Check sheet for the modelled part. Datum: model origin and axes. Units: mm. Give positions to 0.01 mm unless a question says otherwise; leave off trailing zeros. Loops run counter-clockwise (first coordinate to the right, second up) from the corner with the lowest first, then second, coordinate; pieces in that order, holes last. Notation, with made-up numbers: (-10, 45.25) -> (48, 45.25) arc R30 ccw to (48, 78.25) -> close; hole circle Ø8 at (69, 12). An arc over 180 degrees is marked (long way). Answer as CSV lines item,"result". Start each with the question number.
(1) Gauge pin test, flat ends, axial feed: pin 1 Ø1.5 at (y, z) = (214, 5) entering from -X; pin 2 Ø2 at (x, z) = (170, 4) entering from +Y; pin 3 Ø2 at (y, z) = (125.5, 5.5) entering from +X. Record the tip position at first contact, or that the pin passes through.
(2) Material ranges on line 1 (X direction, y = 262, z = 6); line 2 (Y direction, x = 0, z = 3); line 3 (Y direction, x = 20.5, z = 4.5), recorded low to high. Write a range as from..to.
(3) Section check B-B on x = 67. Enter the section's corners in (y, z).
(4) Release check for a two-part mould opening along Y. For faces 1 (the face through (7.917, 143.864, 4.93)), 2 (the face through (193.65, 258.174, 4.93)), 3 (the face through (44, 152, 5)), 4 (the face through (200.4, 252.26, 4.93)) record: pulls with the +Y half, pulls with the -Y half, needs draft (parallel to the pull), parting line crosses it, or undercut.
(5) Section check C-C on y = 219. Enter the section's corners in (x, z), plus the area to 3 significant figures.
(6) Section check A-A on z = 6.25. State how many separate pieces and enclosed holes the cut face has, plus the area to 3 significant figures.
from build123d import *

# Parameters (mm, degrees)
SKETCH_1_R      = 3
SKETCH_1_R_2    = 16
SKETCH_1_R_3    = 3.91899873
SKETCH_1_R_4    = 2
EXTRUDE_1_DEPTH = 10


with BuildPart() as part:
    # 草图1 → 凸台-拉伸1 (new body)
    with BuildSketch(Plane.XY):
        with BuildLine():
            Line((-14, 128), (-6, 0))
            ThreePointArc((-6, 0), (0, -6), (6, 0))
            add(Edge.make_bspline(
                [(6, 0), (1.588652615, 45.680929706), (5.604102499, 79.643200211), (28.004797731, 112.13093391)],
                knots=[0, 0, 0, 0, 0.788155359, 0.788155359, 0.788155359, 0.788155359], degree=3))
            ThreePointArc((28.004797731, 112.13093391), (50.113637924, 128.900750568), (77, 135.767416406))
            ThreePointArc((77, 135.767416406), (157.787149523, 170.485384951), (196.379869136, 249.494896157))
            ThreePointArc((196.379869136, 249.494896157), (200.439238403, 252.311917913), (202, 257))
            Line((202, 257), (202, 262))
            ThreePointArc((202, 262), (194.5, 269.5), (187, 262))
            ThreePointArc((187, 262), (154.781745931, 184.218254069), (77, 152))
            Line((77, 152), (10, 152))
            ThreePointArc((10, 152), (-6.970562748, 144.970562748), (-14, 128))
        make_face()
        Circle(SKETCH_1_R, mode=Mode.SUBTRACT)
        with Locations((10, 128)):
            Circle(SKETCH_1_R_2, mode=Mode.SUBTRACT)
        with Locations((194.5, 262)):
            Circle(SKETCH_1_R_3, mode=Mode.SUBTRACT)
        with Locations((0, 12.5)):
            Circle(SKETCH_1_R_4, mode=Mode.SUBTRACT)
    extrude(amount=EXTRUDE_1_DEPTH)


solid = part.part
Working result:
1,pin 1,"stops at x = 175.61"
1,pin 2,"stops at y = 204.87"
1,pin 3,"stops at x = 45.57"
2,line 1,"x = 187..190.58, 198.42..202"
2,line 2,"y = -6..-3, 3..10.5, 14.5..115.51, 140.49..149.82"
2,line 3,"y = 99.96..115.93, 140.07..152"
3,outline,"(134.54, 0) -> (152, 0) -> (152, 10) -> (134.54, 10) -> close"
4,face 1,"undercut"
4,face 2,"undercut"
4,face 3,"pulls with the +Y half"
4,face 4,"pulls with the -Y half"
5,outline,"(178.25, 0) -> (189.46, 0) -> (189.46, 10) -> (178.25, 10) -> close"
5,area,"112 mm^2"
6,separate pieces,"1"
6,enclosed holes,"4"
6,area,"6,420 mm^2"
